Source: CAD feature listing. Evaluate the final solid. Frame: model axes, mm. Give positions to 0.01 mm unless a question says otherwise; leave off trailing zeros. Write each loop counter-clockwise with the first axis right and the second up, starting at its lowest first coordinate (ties: lowest second). Pieces come first, ordered by that corner, then holes. Notation, with made-up numbers: (44, 31) -> (80, 31) arc R16 ccw to (80, 48) -> close; hole circle Ø11 at (12, -35). An arc over 180 degrees is marked (long way). Use one line per item in the form item = value. Start each with the question number.
(1) Material intervals for line 1 along X through (y, z) = (217, 2.75) (3 decimals); line 2 along X through (y, z) = (167, -0.25) (3 decimals); line 3 along Y through (x, z) = (96, 2), sorted ascending. Write a range as from..to.
(2) Cut plane B-B, the plane x = 91. Output: boundary loops of the cut face in (y, z).
(3) Cut plane A-A, the plane z = 1.5. Output: boundary loops of the cut face in (x, y), and give its area (3 significant figures).
(4) Cut plane C-C, the plane y = 169.5. Output: boundary loops of the cut face in (x, z).
(5) First-contact query: P1, Ø1, axis at x = 21.5, z = 1.5, coming from the +Y side; P2, Ø1.5, axis at x = 87.5, z = -3.5, coming from the -Y side; P3, Ø5, axis at x = 12, z = -1.5, coming from the +Y side; P4, Ø5, axis at y = 143, z = 3, coming from the -X side. Flat tips, straight axial feed; report the tip coordinate or a pass-through.
from build123d import *

# Parameters (mm, degrees)
EXTRUDE_1_DEPTH = 5
CHAMFER_1_SIZE  = 15


with BuildPart() as part:
    # 草图1 → 凸台-拉伸1 (new, symmetric)
    with BuildSketch(Plane.XY):
        Polygon((0, 0), (0, 150), (46, 230), (100, 230), (100, 0), align=None)
    extrude(amount=EXTRUDE_1_DEPTH, both=True)

    # 倒角1
    chamfer_1_edges = [part.edges().sort_by_distance(p)[0] for p in [
        (100, 0, 0),
    ]]
    chamfer(chamfer_1_edges, length=CHAMFER_1_SIZE)


solid = part.part
Geometry says:
q1.line_1 = 38.525..100
q1.line_2 = 9.775..100
q1.line_3 = 11..230
q2.outline = (6, -5) -> (230, -5) -> (230, 5) -> (6, 5) -> close
q3.outline = (0, 0) -> (85, 0) -> (100, 15) -> (100, 230) -> (46, 230) -> (0, 150) -> close
q3.area = 21,000 mm^2
q4.outline = (11.21, -5) -> (100, -5) -> (100, 5) -> (11.21, 5) -> close
q5.P1 = 188.26
q5.P2 = 1.75
q5.P3 = 175.22
q5.P4 = 0
